from build123d import *

# Parameters (mm, degrees)
BOSS_EXTRUDE_DEPTH = 6.4
SKETCH4_W          = 0.6
SKETCH4_H          = 11.237604307
CHAMFER_2_SIZE     = 1.2
FILLET_2_R         = 0.4
LPATTERN1_COUNT    = 13
LPATTERN1_PITCH    = 1.5


with BuildPart() as part:
    # Sketch1 → Boss-Extrude (new body)
    with BuildSketch(Plane(origin=(0, 0, 0), x_dir=(0, 0, -1), z_dir=(1, 0, 0))):
        Polygon((8, 4.618802154), (8, -4.618802154), (0, -9.237604307), (-8, -4.618802154), (-8, 4.618802154), (0, 9.237604307), align=None)
    extrude(amount=BOSS_EXTRUDE_DEPTH)

    # Sketch2 → Boss-Revolve1 (revolve)
    with BuildSketch(Plane.XY, mode=Mode.PRIVATE) as boss_revolve1_sk:
        Polygon((0, 0), (26.4, 0), (26.4, 3.701), (26.4, 5), (0, 5), align=None)
    revolve(boss_revolve1_sk.sketch.rotate(Axis((0, 0, 0), (1, 0, 0)), 90), axis=Axis((0, 0, 0), (1, 0, 0)))

    # Sketch3 → Cut-Revolve1 (revolve, cut)
    with BuildSketch(Plane.XY):
        Polygon((0, 8), (3.601282526, 14.237604307), (3.601282526, 19.237604307), (-10, 19.237604307), (-10, 8), align=None)
    revolve(axis=Axis((0, 0, 0), (1, 0, 0)), mode=Mode.SUBTRACT)

    # Sketch5 → Cut-Revolve2 (revolve, cut)
    with BuildSketch(Plane.XY):
        Polygon((6.4, 8), (2.798717474, 14.237604307), (2.798717474, 19.237604307), (12.798717474, 19.237604307), (12.798717474, 8), align=None)
    revolve(axis=Axis((0, 0, 0), (1, 0, 0)), mode=Mode.SUBTRACT)

    # Sketch4 → Cut-Revolve3 (revolve, cut)
    with BuildSketch(Plane.XY, mode=Mode.PRIVATE) as cut_revolve3_sk:
        with Locations((6.1, 13.618802154)):
            Rectangle(SKETCH4_W, SKETCH4_H)
    revolve(cut_revolve3_sk.sketch.rotate(Axis((0, 0, 0), (1, 0, 0)), 270), axis=Axis((0, 0, 0), (1, 0, 0)), mode=Mode.SUBTRACT)

    # Chamfer 2
    chamfer_2_edges = [part.edges().sort_by_distance(p)[0] for p in [
        (26.4, 0, -5),
    ]]
    chamfer(chamfer_2_edges, length=CHAMFER_2_SIZE)

    # Fillet 2
    fillet_2_edges = [part.edges().sort_by_distance(p)[0] for p in [
        (6.4, 0, -5),
    ]]
    fillet(fillet_2_edges, radius=FILLET_2_R)

    # Sketch6 → Cut-Revolve4 (revolve, cut)
    with BuildSketch(Plane.XY):
        Polygon((7.549978, -3.701), (6.8, -5), (6.8, -6.25), (8.299955999, -6.25), (8.299955999, -5), align=None)
    cut_revolve4 = revolve(axis=Axis((-3.175, 0, 0), (1, 0, 0)), mode=Mode.SUBTRACT)

    # LPattern1: Cut-Revolve4 ×13
    with Locations(*[(i * LPATTERN1_PITCH, 0, 0) for i in range(1, LPATTERN1_COUNT)]):
        add(cut_revolve4, mode=Mode.SUBTRACT)


solid = part.part
Work out the finished part from the listing and answer in its coordinate system (mm). A direction names the side the tool comes from. Coordinates: 2 decimals unless noted, no trailing zeros. Loops run counter-clockwise (first coordinate to the right, second up) from the corner with the lowest first, then second, coordinate; pieces in that order, holes last. Notation, with made-up numbers: (45, -17) -> (84, -17) arc R23 cw to (84, 11) -> close; hole circle Ø11 at (-27, 89.5). An arc over 180 degrees is marked (long way). Answer as CSV lines item,"result".
1) The part is cut by section A-A (x = 3.5). Give the vertices of the cut face in (y, z), and give its area (3 significant figures).
A:
outline,"(-9.24, 0) -> (-4.62, -8) -> (4.62, -8) -> (9.24, 0) -> (4.62, 8) -> (-4.62, 8) -> close"
area,"222 mm²"
2) For faces 1 (the face through (5.8, 4, 7.2)), 2 (the face through (2.859, -6.961, 3.944)), 3 (the face through (6.1, -3.06, -7.39)), determine the directions among +Z, -Z, +X, -X, +Y, -Y from which every point of the face is accessible in a straight line to the end or side of a thin tool.
A:
face 1,"+Z, +X, +Y"
face 2,"+Z, +X, -X, -Y"
face 3,"+X"
3) Straight lines are drawn through the part: probe 1 along X at (y, z) = (-4.25, 5.75); probe 2 along Y at (x, z) = (4, 4); probe 3 along Y at (x, z) = (23, -1.25). For each, find the intervals that lie inside material, in ascending order.
A:
probe 1,"x = 0 to 6.4"
probe 2,"y = -6.93 to 6.93"
probe 3,"y = -4.3 to 4.3"
4) Flat-ended cylindrical pins translate along their axes: pin 1 (4 mm diameter, centred on x = 17.5, y = -0.5, fed in from +Z); pin 2 (4 mm diameter, centred on y = -4, z = -6, fed in from +X); pin 3 (4.5 mm diameter, centred on y = 2.5, z = 6.5, fed in from +X) (3 decimals). Find the tip coordinate at first contact, or state that the pin passes through.
A:
pin 1,"stops at z = 5"
pin 2,"stops at x = 6.45"
pin 3,"stops at x = 24.965"
